For this review, use the dimensioned drawing (mm, ordinates from the lowest corner) and the shaded views. A direction names the side the tool comes from. Coordinates: 2 decimals unless noted, no trailing zeros. Loops run counter-clockwise (first coordinate to the right, second up) from the corner with the lowest first, then second, coordinate; pieces in that order, holes last. Notation, with made-up numbers: (85.5, -34) - (131.5, -34) arc R19 cw to (131.5, -15) - close; hole circle Ø10 at (84.25, -12). An arc over 180 degrees is marked (long way). Answer in a Markdown table with one row per item. Add a question column.
(1) We need section A-A on x = 17. Write out the cut boundary in (y, z).
(2) For line 1 along X through (y, z) = (10, 6.25) (1 decimal); line 2 along Y through (x, z) = (2.75, 4.25) (1 decimal); line 3 along X through (y, z) = (7.25, 8.5), list the stretches that pass through material, from the lowest coordinate up.
(3) Machinability: for the marked faces 1 and 2, which of the approach directions +Z, -Z, +X, -X, +Y, -Y give a long, thin tool a straight path to every point of the face, cutting with its end or side? Answer none if there is none.
(4) For P1, Ø5, axis at y = 7, z = 10, coming from the +X side; P2, Ø2, axis at x = 5, y = 9.5, coming from the +Z side; P3, Ø2, axis at y = 6, z = 3.5, coming from the +X side, all flat-tipped, find the tip position at first contact; note any pin that passes through.
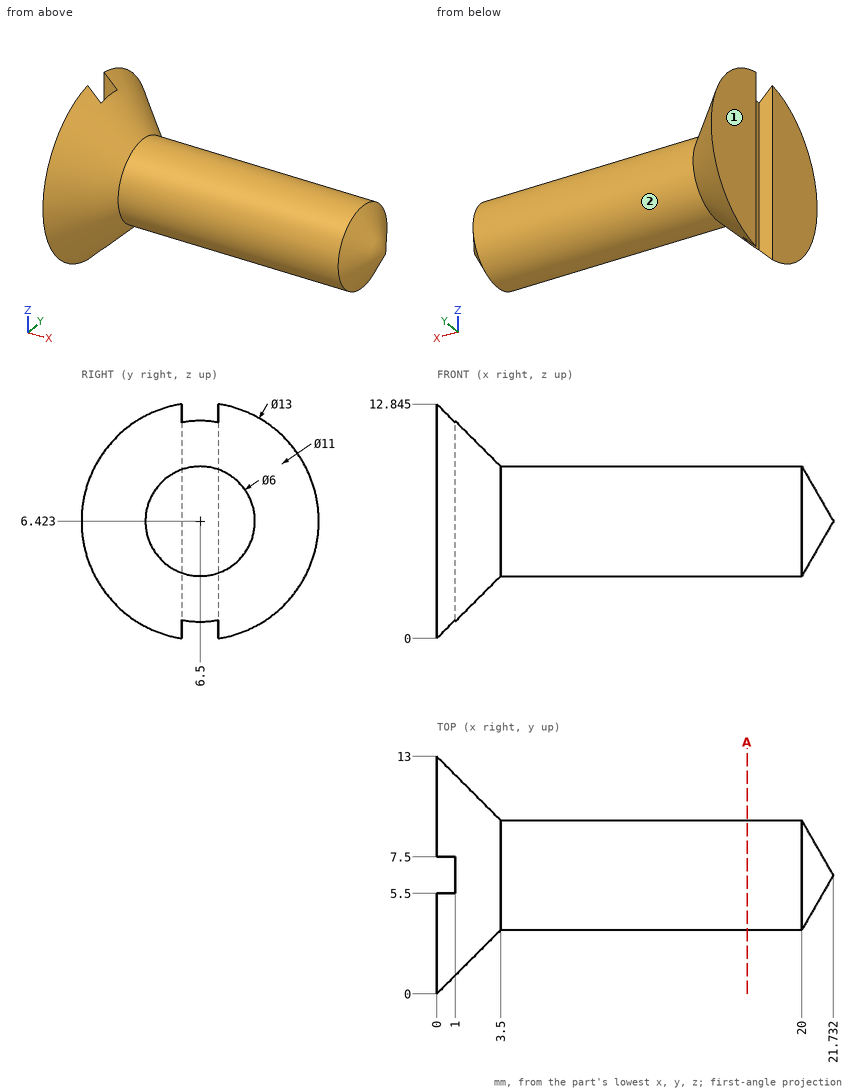
Outcome:
| question | item | result |
|---|---|---|
| 1 | outline | circle Ø6 at (6.5, 6.42) |
| 2 | line 1 | 0 to 3 |
| 2 | line 2 | 3.4 to 9.6 |
| 2 | line 3 | 1 to 20.46 |
| 3 | face 1 | +Z, -Z, -X, +Y, -Y |
| 3 | face 2 | +X |
| 4 | P1 | x = 21.09 |
| 4 | P2 | z = 8.66 |
| 4 | P3 | x = 20.6 |
